from build123d import *

# Parameters (mm, degrees)
SKETCH1_W           = 20
SKETCH1_H           = 30
BOSS_EXTRUDE1_DEPTH = 10
CHAMFER1_SIZE       = 10
SKETCH2_R           = 1.584264685
BOSS_EXTRUDE2_DEPTH = 10


with BuildPart() as part:
    # Sketch1 → Boss-Extrude1 (new body)
    with BuildSketch(Plane(origin=(0, 0, 0), x_dir=(1, 0, 0), z_dir=(0, 1, 0))):
        with Locations((10, -15)):
            Rectangle(SKETCH1_W, SKETCH1_H)
    extrude(amount=BOSS_EXTRUDE1_DEPTH)

    # Chamfer1
    chamfer1_edges = [part.edges().sort_by_distance(p)[0] for p in [
        (20, 5, 30),
    ]]
    chamfer(chamfer1_edges, length=CHAMFER1_SIZE)

    # Sketch2 → Boss-Extrude2 (add)
    with BuildSketch(Plane(origin=(20, 0, 20), x_dir=(0.7071067811865487, 0, -0.7071067811865465), z_dir=(0.7071067811865465, 0, 0.7071067811865487))):
        with Locations((-7.203605768, 5.360257058)):
            Circle(SKETCH2_R)
    extrude(amount=BOSS_EXTRUDE2_DEPTH)


solid = part.part
Can you work these out from the model? Positions are in its coordinate system, mm. A direction names the side the tool comes from. Round coordinates to 2 decimals unless told otherwise and drop trailing zeros. Order: outer loops, then holes, each group sorted by start corner. A loop starts at its lowest first (then second) coordinate and runs counter-clockwise, first axis right, second up. Notation, with made-up numbers: (63.5, -1.75) - (105.5, -1.75) arc R10 cw to (105.5, 5.25) - close; hole circle Ø1 at (39.5, 77.25). An arc over 180 degrees is marked (long way). Answer in a Markdown table with one row per item.
(1) Suppose I cut it at C-C, the plane z = 23. Please give me the cut outline in (x, y), plus the area to 3 significant figures.
From the geometry:
| item | result |
|---|---|
| outline | (0, 0) - (17, 0) - (17, 10) - (0, 10) - close |
| area | 170 mm2 |
(2) If we mould it in two halves opening along X, with no side actions, what happens to faces 3 (the face through (10, 0, 15)), 4 (the face through (16.2, 4.9, 23.8)), 5 (the face through (20, 5, 10))? For each: released by +X, released by -X, zero draft, split by the parting line, or undercut.
From the geometry:
| item | result |
|---|---|
| face 3 | zero draft |
| face 4 | undercut |
| face 5 | released by +X |
(3) Please list where these lines run through material, in increasing order: L1, parallel to Z at x = 10, y = 6; L2, parallel to X at y = 7.75, z = 8; L3, parallel to X at y = 6.5, z = 28. Write a range as from..to.
From the geometry:
| item | result |
|---|---|
| L1 | z = 0..30 |
| L2 | x = 0..20 |
| L3 | x = 0..12, 16.26..19.37 |
(4) Suppose I cut it at B-B, the plane x = 11.25. Please give me the cut outline in (y, z), plus the area to 4 significant figures.
From the geometry:
| item | result |
|---|---|
| outline | (0, 0) - (10, 0) - (10, 28.75) - (0, 28.75) - close |
| area | 287.5 mm2 |
(5) For P1, Ø5, axis at y = 4.5, z = 5, coming from the +X side; P2, Ø5, axis at x = 7, y = 4.5, coming from the +Z side, each with a flat end and sliding along its axis, tell me the tip position at first contact or that it passes through.
From the geometry:
| item | result |
|---|---|
| P1 | stops at x = 20 |
| P2 | stops at z = 30 |
(6) Suppose I cut it at A-A, the plane y = 3. Please give me the cut outline in (x, z), plus the area to 3 significant figures.
From the geometry:
| item | result |
|---|---|
| outline | (0, 0) - (20, 0) - (20, 20) - (10, 30) - (0, 30) - close |
| area | 550 mm2 |
(7) Which directions (+Z, -Z, +X, -X, +Y, -Y) give clear straight access to the entire face, cutting with the end or side of a thin tool? Please do faces 1 (the face through (21.96, 5.38, 32.18)), 2 (the face through (5, 5, 30)).
From the geometry:
| item | result |
|---|---|
| face 1 | +Z, +X, +Y, -Y |
| face 2 | +Z, -X, +Y, -Y |
